Geometry check sheet. Reference: the model listing, model coordinates, mm. Face numbers are marked on the shaded views. A direction names the side the tool comes from. Give positions to 0.01 mm unless a question says otherwise; leave off trailing zeros. Loops run counter-clockwise (first coordinate to the right, second up) from the corner with the lowest first, then second, coordinate; pieces in that order, holes last. Notation, with made-up numbers: (-15, 56.25) - (0, 56.25) arc R19 ccw to (0, 68.25) - close; hole circle Ø4 at (81, -30.75). An arc over 180 degrees is marked (long way). One line per question, with ' | ' between items. Start each with the question number.
from build123d import *

# Parameters (mm, degrees)
BOSS_EXTRUDE1_DEPTH = 207.5


with BuildPart() as part:
    # Sketch1 → Boss-Extrude1 (new body)
    with BuildSketch(Plane.XY):
        with BuildLine():
            Line((-290, 140), (-36.538558432, 189.000486104))
            ThreePointArc((-36.538558432, 189.000486104), (192.5, 0), (-36.538558432, -189.000486104))
            Line((-36.538558432, -189.000486104), (-290, -140))
            Line((-290, -140), (-286.583407523, -122.327227273))
            Line((-286.583407523, -122.327227273), (-33.121965956, -171.327713378))
            ThreePointArc((-33.121965956, -171.327713378), (174.5, 0), (-33.121965956, 171.327713378))
            Line((-33.121965956, 171.327713378), (-286.583407523, 122.327227273))
            Line((-286.583407523, 122.327227273), (-290, 140))
        make_face()
    extrude(amount=BOSS_EXTRUDE1_DEPTH)


solid = part.part
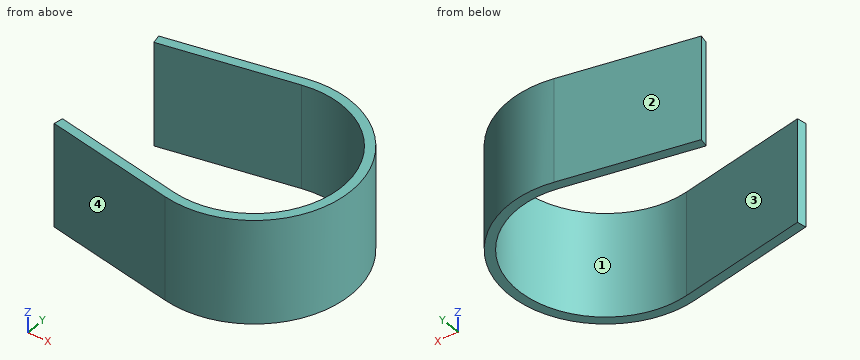
(1) Depth check by flat-ended pin: pin 1 Ø3 at (x, z) = (-51, 132.5) entering from +Y; pin 2 Ø2 at (y, z) = (-101.5, 100) entering from +X; pin 3 Ø12 at (y, z) = (-152, 74) entering from +X. Enter the tip coordinate at first touch or a pass-through.
(2) Section check B-B, the plane z = 18. Record the boundary of the cut face in (x, y), and give its area (3 significant figures).
(3) Material ranges on line 1 (Y direction, x = 0, z = 111.5); line 2 (Y direction, x = -70.5, z = 25); line 3 (X direction, y = 0, z = 112), recorded low to high.
(4) Tool access check on the marked faces 3 and 4. Record the directions out of +Z, -Z, +X, -X, +Y, -Y that give a thin tool (end or side, any length) a straight path to the whole face; none if there is none.
(5) Section check A-A, the plane x = 0. Record the boundary of the cut face in (y, z), and give its area (3 significant figures).
(6) Section check D-D, the plane x = -184.5. Record the boundary of the cut face in (y, z).
(7) Section check C-C, the plane y = 0. Record the boundary of the cut face in (x, z), and give its area (4 significant figures).
(8) Mould release check, pull along X, two halves, no side actions. Record for the marked faces 1 and 2: pulls with the +X half, pulls with the -X half, needs draft (parallel to the pull), parting line crosses it, or undercut.
Numbers:
1) pin 1: y = 186.49 | pin 2: x = 164.18 | pin 3: x = 125.46
2) outline: (-290, -140) - (-36.54, -189) arc R192.5 ccw (long way) to (-36.54, 189) - (-290, 140) - (-286.58, 122.33) - (-33.12, 171.33) arc R174.5 cw (long way) to (-33.12, -171.33) - (-286.58, -122.33) - close | area: 20,900 mm^2
3) line 1: -192.5 to -174.5, 174.5 to 192.5 | line 2: -182.43 to -164.1, 164.1 to 182.43 | line 3: 174.5 to 192.5
4) face 3: +Z, -Z | face 4: +Z, -Z, -X, -Y
5) outline: (-192.5, 0) - (-174.5, 0) - (-174.5, 207.5) - (-192.5, 207.5) - close; (174.5, 0) - (192.5, 0) - (192.5, 207.5) - (174.5, 207.5) - close | area: 7,470 mm^2
6) outline: (-160.4, 0) - (-142.06, 0) - (-142.06, 207.5) - (-160.4, 207.5) - close; (142.06, 0) - (160.4, 0) - (160.4, 207.5) - (142.06, 207.5) - close
7) outline: (174.5, 0) - (192.5, 0) - (192.5, 207.5) - (174.5, 207.5) - close | area: 3,735 mm^2
8) face 1: undercut | face 2: pulls with the -X half
